from build123d import *

# Parameters (mm, degrees)
ARCHED_BODY_60_DEPTH         = 60
POCKET_A_STEP_CUT_5_DEPTH    = 5
POCKET_A_CUT_12_DEPTH        = 12
POCKET_B_STEP_CUT_5_DEPTH    = 5
POCKET_B_SKETCH_W            = 15
POCKET_B_SKETCH_H            = 40
POCKET_B_CUT_12_DEPTH        = 12
TOP_HALF_ROUND_CUT_40_DEPTH  = 40
TOP_PAD_SKETCH_W             = 30
TOP_PAD_SKETCH_H             = 20
TOP_PAD_5_DEPTH              = 5
TOP_HALF_ROUND_BOSS_20_DEPTH = 20


with BuildPart() as part:
    # Arched Body Profile Sketch → Arched Body 60 (new body)
    with BuildSketch(Plane.XY):
        with BuildLine():
            Line((0, 0), (25, 0))
            ThreePointArc((25, 0), (45, 20), (65, 0))
            Line((65, 0), (90, 0))
            Line((90, 0), (90, 10))
            Line((90, 10), (75, 40))
            Line((75, 40), (70, 40))
            Line((70, 40), (70, 70))
            Line((70, 70), (60, 70))
            ThreePointArc((60, 70), (45, 85), (30, 70))
            Line((30, 70), (20, 70))
            Line((20, 70), (20, 40))
            Line((20, 40), (15, 40))
            Line((15, 40), (0, 10))
            Line((0, 10), (0, 0))
        make_face()
    extrude(amount=ARCHED_BODY_60_DEPTH)

    # Pocket A Step Sketch → Pocket A Step Cut 5 (cut)
    with BuildSketch(Plane.ZY.offset(-20)):
        Polygon((30, 70), (10, 70), (10, 40), (50.046888812, 40), (50.046888812, 70), align=None)
    extrude(amount=-POCKET_A_STEP_CUT_5_DEPTH, mode=Mode.SUBTRACT)

    # Pocket A Sketch → Pocket A Cut 12 (cut)
    with BuildSketch(Plane(origin=(0, 40, 0), x_dir=(1, 0, 0), z_dir=(0, 1, 0))):
        Polygon((20, -10), (15, -10), (5, -10), (5, -50), (15, -50), (25, -50.046888812), (25, -10), align=None)
    extrude(amount=-POCKET_A_CUT_12_DEPTH, mode=Mode.SUBTRACT)

    # Pocket B Step Sketch → Pocket B Step Cut 5 (cut)
    with BuildSketch(Plane(origin=(70, 0, 0), x_dir=(0, 0, -1), z_dir=(1, 0, 0))):
        Polygon((-30, 70), (-50, 70), (-50, 40), (-10, 40), (-10, 70), align=None)
    extrude(amount=-POCKET_B_STEP_CUT_5_DEPTH, mode=Mode.SUBTRACT)

    # Pocket B Sketch → Pocket B Cut 12 (cut)
    with BuildSketch(Plane(origin=(0, 40, 0), x_dir=(1, 0, 0), z_dir=(0, 1, 0))):
        with Locations((72.5, -30)):
            Rectangle(POCKET_B_SKETCH_W, POCKET_B_SKETCH_H)
    extrude(amount=-POCKET_B_CUT_12_DEPTH, mode=Mode.SUBTRACT)

    # Top Half-Round Cut Sketch → Top Half-Round Cut 40 (cut)
    with BuildSketch(Plane(origin=(0, 0, 0), x_dir=(-1, 0, 0), z_dir=(0, 0, -1))):
        with BuildLine():
            Line((-60, 70), (-30, 70))
            ThreePointArc((-30, 70), (-45, 85), (-60, 70))
        make_face()
    extrude(amount=-TOP_HALF_ROUND_CUT_40_DEPTH, mode=Mode.SUBTRACT)

    # Top Pad Sketch → Top Pad 5 (add)
    with BuildSketch(Plane(origin=(0, 70, 0), x_dir=(1, 0, 0), z_dir=(0, 1, 0))):
        with Locations((45, -30)):
            Rectangle(TOP_PAD_SKETCH_W, TOP_PAD_SKETCH_H)
    extrude(amount=TOP_PAD_5_DEPTH)

    # Top Half-Round Boss Sketch → Top Half-Round Boss 20 (add)
    with BuildSketch(Plane(origin=(0, 0, 0), x_dir=(-1, 0, 0), z_dir=(0, 0, -1))):
        with BuildLine():
            Line((-60, 70), (-30, 70))
            ThreePointArc((-30, 70), (-45, 85), (-60, 70))
        make_face()
    extrude(amount=-TOP_HALF_ROUND_BOSS_20_DEPTH)


solid = part.part
Could you check a few things on this model? Use its own coordinates, in mm. A direction names the side the tool comes from. Give positions to 0.01 mm unless a question says otherwise; leave off trailing zeros. Order: outer loops, then holes, each group sorted by start corner. A loop starts at its lowest first (then second) coordinate and runs counter-clockwise, first axis right, second up.
1. Suppose I cut it at D-D (y = 59.5). List the corners of the cut face in (x, z) for me.
2. Suppose I cut it at B-B (y = 7.5). List the corners of the cut face in (x, z) for me.
3. We'd pull the mould along Z, two halves only. Please class faces 1 (the flat face through (45, 75, 30)), 2 (the flat face through (44, 34, 60)), 3 (the flat face through (30, 72, 30)): pulls with the +Z half, pulls with the -Z half, needs draft (parallel to the pull), parting line crosses it, or undercut.
4. Suppose I cut it at C-C (x = 11.5). List the corners of the cut face in (y, z) for me.
5. Suppose I cut it at A-A (z = 12). List the corners of the cut face in (x, y) for me.
6. I need wall thicknesses on L1, parallel to X at y = 50, z = 21.5; L2, parallel to Y at x = 79.5, z = 18; L3, parallel to X at y = 29, z = 40.5. Which ranges of each line are inside material? Lowest first, please.
7. Will these pins go through, and if not, where does the flat tip stop? P1, Ø1, axis at x = 63, y = 17.5, coming from the -Z side; P2, Ø12, axis at y = 47.5, z = 25, coming from the -X side; P3, Ø1.5, axis at x = 55.5, z = 52.5, coming from the +Y side; P4, Ø1, axis at x = 41, z = 52.5, coming from the -Y side.
8. For faces 4 (the flat face through (90, 5, 30)), 5 (the flat face through (22, 55, 50.047)), 6 (the cylindrical face through (45, 85, 50)), 7 (the flat face through (45, 79, 40)), 8 (the flat face through (73, 40, 5)), which set-ups out of +Z, -Z, +X, -X, +Y, -Y let a thin tool reach every point of the face, with its end or its side?
Solved:
1. outline: (20, 0) - (70, 0) - (70, 10) - (65, 10) - (65, 50) - (70, 50) - (70, 60) - (20, 60) - (20, 50.05) - (25, 50.05) - (25, 10) - (20, 10) - close
2. outline: (0, 0) - (26.46, 0) - (26.46, 60) - (0, 60) - close; (63.54, 0) - (90, 0) - (90, 60) - (63.54, 60) - close
3. face 1: undercut
3. face 2: pulls with the +Z half
3. face 3: needs draft
4. outline: (0, 0) - (33, 0) - (33, 10) - (28, 10) - (28, 50) - (33, 50) - (33, 60) - (0, 60) - close
5. outline: (0, 0) - (25, 0) arc R20 cw to (65, 0) - (90, 0) - (90, 10) - (80, 30) - (80, 28) - (65, 28) - (65, 70) - (60, 70) arc R15 ccw to (30, 70) - (25, 70) - (25, 28) - (9, 28) - (0, 10) - close
6. L1: x = 25 to 65
6. L2: y = 0 to 28
6. L3: x = 25 to 65, 80 to 80.5
7. P1: stops at z = 0
7. P2: stops at x = 25
7. P3: stops at y = 81.4
7. P4: stops at y = 19.49
8. face 4: +Z, -Z, +X, +Y, -Y
8. face 5: -X, +Y
8. face 6: +Z, +Y
8. face 7: +X, -X, +Y
8. face 8: +Z, -Z, +X, +Y
